The listing builds one solid part. Answer for the finished solid, in the listing's coordinates (mm). Face numbers are marked on the shaded views. A direction names the side the tool comes from. Give positions to 0.01 mm unless a question says otherwise; leave off trailing zeros. Order: outer loops, then holes, each group sorted by start corner. A loop starts at its lowest first (then second) coordinate and runs counter-clockwise, first axis right, second up. Notation, with made-up numbers: (70, -21.5) - (128, -21.5) arc R12 cw to (128, -6.5) - close; hole circle Ø1 at (-32, -1.75). An arc over 180 degrees is marked (long way). Answer in a Markdown table with one row per item.
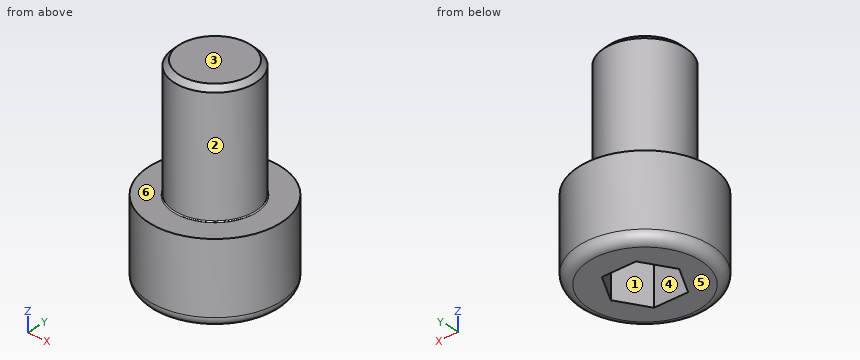
from build123d import *

# Parameters (mm, degrees)
SKETCH_1_R          = 6.5
EXTRUDE_1_DEPTH     = 8
SKETCH_2_R          = 4
EXTRUDE_2_DEPTH     = 12
CUT_EXTRUDE_1_DEPTH = 4
FILLET_1_R          = 0.1
CHAMFER_1_SIZE      = 0.5
FILLET_2_R          = 1


with BuildPart() as part:
    # 草图1 → 凸台-拉伸1 (new body)
    with BuildSketch(Plane.XY):
        Circle(SKETCH_1_R)
    extrude(amount=EXTRUDE_1_DEPTH)

    # 草图2 → 凸台-拉伸2 (add)
    with BuildSketch(Plane.XY.offset(8)):
        Circle(SKETCH_2_R)
    extrude(amount=EXTRUDE_2_DEPTH)

    # 草图3 → 切除-拉伸1 (cut)
    with BuildSketch(Plane(origin=(0, 0, 0), x_dir=(-1, 0, 0), z_dir=(0, 0, -1))):
        Polygon((1.732050808, -3), (3.464101615, 0), (1.732050808, 3), (-1.732050808, 3), (-3.464101615, 0), (-1.732050808, -3), align=None)
    extrude(amount=-CUT_EXTRUDE_1_DEPTH, mode=Mode.SUBTRACT)

    # 圆角1
    fillet_1_edges = [part.edges().sort_by_distance(p)[0] for p in [
        (-4, 0, 8),
    ]]
    fillet(fillet_1_edges, radius=FILLET_1_R)

    # 倒角1
    chamfer_1_edges = [part.edges().sort_by_distance(p)[0] for p in [
        (-4, 0, 20),
    ]]
    chamfer(chamfer_1_edges, length=CHAMFER_1_SIZE)

    # 圆角2
    fillet_2_edges = [part.edges().sort_by_distance(p)[0] for p in [
        (-6.5, 0, 0),
    ]]
    fillet(fillet_2_edges, radius=FILLET_2_R)


solid = part.part
Item 1: Determine the mould class of the marked faces 1, 2, 3 and 4 for opening direction Y: pulls with the +Y half, pulls with the -Y half, needs draft (parallel to the pull), parting line crosses it, or undercut.
Answer block:
| item | result |
|---|---|
| face 1 | undercut |
| face 2 | parting line crosses it |
| face 3 | needs draft |
| face 4 | undercut |
Item 2: Which of the six approach directions +Z, -Z, +X, -X, +Y, -Y give full straight-line access (tool end or side, diameter ignored) to the marked faces 5 and 6?
Answer block:
| item | result |
|---|---|
| face 5 | -Z, +X, -X, +Y, -Y |
| face 6 | +Z |
Item 3: Consider line 1 (Z direction, x = 3, y = 0.25); line 2 (Z direction, x = 2.25, y = 4.5); line 3 (Y direction, x = 0, z = 3.5). Determine where each line is inside the solid, lowest interval first.
Answer block:
| item | result |
|---|---|
| line 1 | 4 to 20 |
| line 2 | 0 to 8 |
| line 3 | -6.5 to -3, 3 to 6.5 |
Item 4: Find section A-A on x = 0. Write down the section's boundary in (y, z).
Answer block:
| item | result |
|---|---|
| outline | (-6.5, 1) arc R1 ccw to (-5.5, 0) - (-3, 0) - (-3, 4) - (3, 4) - (3, 0) - (5.5, 0) arc R1 ccw to (6.5, 1) - (6.5, 8) - (4.1, 8) arc R0.1 cw to (4, 8.1) - (4, 19.5) - (3.5, 20) - (-3.5, 20) - (-4, 19.5) - (-4, 8.1) arc R0.1 cw to (-4.1, 8) - (-6.5, 8) - close |
Item 5: Find section B-B on z = 10.25. Write down the section's boundary in (x, y).
Answer block:
| item | result |
|---|---|
| outline | circle Ø8 at (0, 0) |
Item 6: Each of these flat-tipped pins is pushed along its axis until it touches: P1, Ø1, axis at y = -4, z = 16.5, coming from the +X side; P2, Ø6, axis at x = 2.5, z = 16.5, coming from the +Y side; P3, Ø4, axis at y = 4.5, z = 5.5, coming from the -X side. Where does it stop, or does it pass through?
Answer block:
| item | result |
|---|---|
| P1 | x = 1.94 |
| P2 | y = 4 |
| P3 | x = -6 |
